For this review, take the finished solid that the model builds, in its own axes (mm). Face numbers are marked on the shaded views. A direction names the side the tool comes from. Give positions to 0.01 mm unless a question says otherwise; leave off trailing zeros. Order: outer loops, then holes, each group sorted by start corner. A loop starts at its lowest first (then second) coordinate and runs counter-clockwise, first axis right, second up. Notation, with made-up numbers: (15, 59) - (60, 59) arc R21 cw to (60, 93) - close; hole circle Ø5 at (37.5, 83). An arc over 180 degrees is marked (long way). Put each result on its own line as item: value. Start each with the question number.
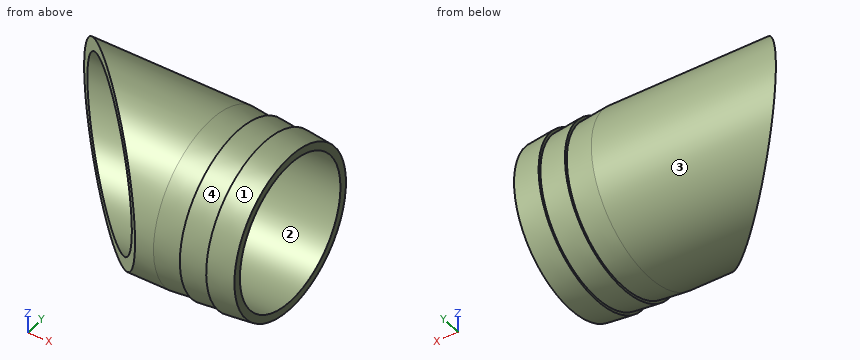
```python
from build123d import *

# Parameters (mm, degrees)
CUT_EXTRUDE1_DEPTH      = 110.473741144
CUT_EXTRUDE1_DEPTH_BACK = 110.473741144


with BuildPart() as part:
    # Sketch1 → Revolve1 (revolve)
    with BuildSketch(Plane.XY, mode=Mode.PRIVATE) as revolve1_sk:
        Polygon((0, 27.5), (0, 31.5), (70, 31.5), (80, 30.5), (80, 31.5), (90, 30.5), (90, 31.5), (100, 30.5), (100, 27.5), align=None)
    revolve(revolve1_sk.sketch.rotate(Axis((0, 0, 0), (1, 0, 0)), 90), axis=Axis((0, 0, 0), (1, 0, 0)))

    # Sketch2 → Cut-Extrude1 (cut, two sides: drawn at the far end of the back side and taken through both)
    with BuildSketch(Plane.XY.offset(-CUT_EXTRUDE1_DEPTH_BACK)):
        Polygon((-199.7384521, 231.2384521), (0, 31.5), (96.333692144, -64.833692144), (296.072144244, -264.572144244), (-103.404759956, -664.049048445), (-599.2153563, -168.2384521), align=None)
    extrude(amount=CUT_EXTRUDE1_DEPTH + CUT_EXTRUDE1_DEPTH_BACK, mode=Mode.SUBTRACT)


solid = part.part
```
1. Clearance check with flat-ended pins moving along their axes: pin 1 (1 mm diameter, centred on x = 62, z = 21.5, fed in from -Y); pin 2 (4 mm diameter, centred on x = 79.5, y = 21.5, fed in from -Z); pin 3 (4 mm diameter, centred on x = 29.5, y = -0.5, fed in from +Z). State where each tip first meets the part, or that it passes through.
2. The part is to be moulded in two halves that separate along Z. For the marked faces 1 and 2, say which applies: released by +Z, released by -Z, zero draft, split by the parting line, or undercut.
3. Wall thickness on line 1 (Y direction, x = 67, z = 0); line 2 (Y direction, x = 40, z = 0); line 3 (Y direction, x = 92, z = 16): over which ranges is each line inside the solid? List them lowest first. Write a range as from..to.
4. Add section B-B, the plane z = 0. Give the boundary of the cut face in (x, y).
5. Add section D-D, the plane x = 9. Give the boundary of the cut face in (y, z).
6. Add section C-C, the plane x = 76.5. Give the boundary of the cut face in (y, z).
7. Add section A-A, the plane y = 0. Give the boundary of the cut face in (x, z), then the cut area to 3 significant figures.
8. Tool access review of the marked faces 3 and 4: name each direction out of +Z, -Z, +X, -X, +Y, -Y from which nothing blocks a thin tool from reaching the whole face with its end or side.
Found:
1. pin 1: stops at y = -23.48
1. pin 2: stops at z = -24.69
1. pin 3: stops at z = 31.5
2. face 1: split by the parting line
2. face 2: undercut
3. line 1: y = -31.5..-27.5, 27.5..31.5
3. line 2: y = 27.5..31.5
3. line 3: y = -26.9..-22.37, 22.37..26.9
4. outline: (0, 31.5) - (4, 27.5) - (100, 27.5) - (100, 30.5) - (90, 31.5) - (90, 30.5) - (80, 31.5) - (80, 30.5) - (70, 31.5) - close; (59, -27.5) - (63, -31.5) - (70, -31.5) - (80, -30.5) - (80, -31.5) - (90, -30.5) - (90, -31.5) - (100, -30.5) - (100, -27.5) - close
5. outline: (22.5, -22.05) arc R31.5 ccw to (22.5, 22.05) - (22.5, 15.81) arc R27.5 cw to (22.5, -15.81) - close
6. outline: circle Ø61.7 at (0, 0); hole circle Ø55 at (0, 0)
7. outline: (31.5, -31.5) - (70, -31.5) - (80, -30.5) - (80, -31.5) - (90, -30.5) - (90, -31.5) - (100, -30.5) - (100, -27.5) - (31.5, -27.5) - close; (31.5, 27.5) - (100, 27.5) - (100, 30.5) - (90, 31.5) - (90, 30.5) - (80, 31.5) - (80, 30.5) - (70, 31.5) - (31.5, 31.5) - close
7. area: 518 mm^2
8. face 3: +X, -X
8. face 4: none
